```python
from build123d import *

# Parameters (mm, degrees)
EXTRUDE_1_DEPTH     = 16
SKETCH_2_R          = 1.65
CUT_EXTRUDE_1_DEPTH = 7.5


with BuildPart() as part:
    # 草图1 → 凸台-拉伸1 (new, symmetric)
    with BuildSketch(Plane.XY):
        Polygon((0, 0), (28, 0), (28, 3), (3, 3), (3, 65), (0, 65), align=None)
    extrude(amount=EXTRUDE_1_DEPTH, both=True)

    # 草图2 → 切除-拉伸1 (cut, symmetric)
    with BuildSketch(Plane(origin=(0, 0, 0), x_dir=(1, 0, 0), z_dir=(0, 1, 0))):
        with Locations(Location((6, 0, 0), (0, 0, 270))):
            Circle(SKETCH_2_R)
        with Locations(Location((22, 0, 0), (0, 0, 270))):
            Circle(SKETCH_2_R)
    extrude(amount=CUT_EXTRUDE_1_DEPTH, both=True, mode=Mode.SUBTRACT)


solid = part.part
```
The listing builds one solid part. Answer for the finished solid, in the listing's coordinates (mm). A direction names the side the tool comes from. Give positions to 0.01 mm unless a question says otherwise; leave off trailing zeros. Order: outer loops, then holes, each group sorted by start corner. A loop starts at its lowest first (then second) coordinate and runs counter-clockwise, first axis right, second up.
Item 1: For a pull along X with two mould halves and no side action, classify faces 1 (the face through (0, 33, 0)), 2 (the face through (4.4, 1.5, -0.4)), 3 (the face through (2.5, 25.4, -16)) as pulls with the +X half, pulls with the -X half, needs draft (parallel to the pull), parting line crosses it, or undercut.
From the geometry:
face 1: pulls with the -X half
face 2: undercut
face 3: needs draft
Item 2: The part is cut by section B-B, the plane z = 10. Give the vertices of the cut face in (x, y).
From the geometry:
outline: (0, 0) - (28, 0) - (28, 3) - (3, 3) - (3, 65) - (0, 65) - close
Item 3: Given pin 1 Ø2 at (x, z) = (11, -8.5) entering from +Y; pin 2 Ø5 at (x, y) = (7, 49.5) entering from -Z; pin 3 Ø9.5 at (y, z) = (27, -6.5) entering from +X, each flat-ended and moving along its own axis, determine where each tip first touches the part or whether it passes through.
From the geometry:
pin 1: stops at y = 3
pin 2: passes through
pin 3: stops at x = 3
Item 4: The part is cut by section A-A, the plane x = 22. Give the vertices of the cut face in (y, z), and give its area (3 significant figures).
From the geometry:
outline: (0, -16) - (3, -16) - (3, -1.65) - (0, -1.65) - close; (0, 1.65) - (3, 1.65) - (3, 16) - (0, 16) - close
area: 86.1 mm2
Item 5: Which of the six approach directions +Z, -Z, +X, -X, +Y, -Y give full straight-line access (tool end or side, diameter ignored) to faces 4 (the face through (16, 3, 0)), 5 (the face through (23.636, 1.521, -0.215))?
From the geometry:
face 4: +Z, -Z, +X, +Y
face 5: +Y, -Y
Item 6: The part is cut by section C-C, the plane x = 25.5. Give the vertices of the cut face in (y, z).
From the geometry:
outline: (0, -16) - (3, -16) - (3, 16) - (0, 16) - close
Item 7: Find the intervals of material crossed by probe 1 along X at (y, z) = (1.2, 0); probe 2 along Z at (x, y) = (6, 1.65); probe 3 along Y at (x, z) = (17.5, -11.5), in increasing order.
From the geometry:
probe 1: x = 0 to 4.35, 7.65 to 20.35, 23.65 to 28
probe 2: z = -16 to -1.65, 1.65 to 16
probe 3: y = 0 to 3
